Here's how the part is built. I have some questions about the finished solid (model axes, mm). A direction names the side the tool comes from. Give positions to 0.01 mm unless a question says otherwise; leave off trailing zeros. Write each loop counter-clockwise with the first axis right and the second up, starting at its lowest first coordinate (ties: lowest second). Pieces come first, ordered by that corner, then holes. Notation, with made-up numbers: (-5.75, -17) -> (20.25, -17) arc R3 cw to (20.25, -13) -> close; hole circle Ø5 at (30, -20). An arc over 180 degrees is marked (long way). Answer as CSV lines item,"result". Start each with the question number.
from build123d import *

# Parameters (mm, degrees)
SKETCH_1_W          = 30
SKETCH_1_H          = 30
SKETCH_1_W_2        = 26
SKETCH_1_H_2        = 26
EXTRUDE_1_DEPTH     = 520
SKETCH_3_R          = 3.3
CUT_EXTRUDE_1_DEPTH = 636


with BuildPart() as part:
    # 草图1 → 凸台-拉伸1 (new, symmetric)
    with BuildSketch(Plane.XY):
        Rectangle(SKETCH_1_W, SKETCH_1_H)
        Rectangle(SKETCH_1_W_2, SKETCH_1_H_2, mode=Mode.SUBTRACT)
    extrude(amount=EXTRUDE_1_DEPTH, both=True)

    # 草图3 → 切除-拉伸1 (cut)
    with BuildSketch(Plane(origin=(0, 15, 0), x_dir=(1, 0, 0), z_dir=(0, 1, 0))):
        with Locations(Location((0, 360, 0), (0, 0, 270))):
            Circle(SKETCH_3_R)
        with Locations(Location((0, 180, 0), (0, 0, 270))):
            Circle(SKETCH_3_R)
        with Locations(Location((0, 0, 0), (0, 0, 270))):
            Circle(SKETCH_3_R)
        with Locations(Location((0, -180, 0), (0, 0, 270))):
            Circle(SKETCH_3_R)
        with Locations(Location((0, -360, 0), (0, 0, 270))):
            Circle(SKETCH_3_R)
    extrude(amount=-CUT_EXTRUDE_1_DEPTH, mode=Mode.SUBTRACT)


solid = part.part
Item 1: We'd pull the mould along Y, two halves only. Please class faces 3 (the face through (-15, 0, 7)), 4 (the face through (0, -13, 7)), 5 (the face through (0, 15, 7)): released by +Y, released by -Y, zero draft, split by the parting line, or undercut.
Item 2: For faces 1 (the face through (0, -15, 7)), 2 (the face through (13, 0, 7)), which set-ups out of +Z, -Z, +X, -X, +Y, -Y let a thin tool reach every point of the face, with its end or its side?
Item 3: If I drill on line 1 (X direction, y = -12.5, z = -347); line 2 (X direction, y = 13.65, z = 0), over which ranges is the centre line in solid material (lowest first)? Write a range as [from, to].
Item 4: If we section it at A-A (y = 2): Please give me the cut outline in (x, z).
Item 5: If we section it at B-B (z = 444.5): Please give me the cut outline in (x, y), and give its area (3 significant figures).
Final values:
1,face 3,"zero draft"
1,face 4,"undercut"
1,face 5,"released by +Y"
2,face 1,"+Z, -Z, +X, -X, -Y"
2,face 2,"+Z, -Z"
3,line 1,"[-15, -13], [13, 15]"
3,line 2,"[-15, -3.3], [3.3, 15]"
4,outline,"(-15, -520) -> (-13, -520) -> (-13, 520) -> (-15, 520) -> close; (13, -520) -> (15, -520) -> (15, 520) -> (13, 520) -> close"
5,outline,"(-15, -15) -> (15, -15) -> (15, 15) -> (-15, 15) -> close; hole (-13, -13) -> (13, -13) -> (13, 13) -> (-13, 13) -> close"
5,area,"224 mm2"
